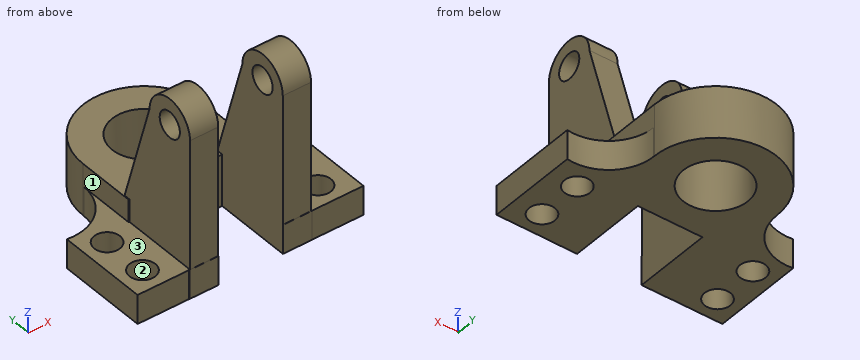
from build123d import *

# Parameters (mm, degrees)
HUB_BODY_SKETCH_R             = 20
HUB_BODY_DEPTH                = 32
MOUNTING_PLATE_DEPTH          = 18
SIDE_WEB_SKETCH_W             = 18
SIDE_WEB_SKETCH_H             = 48.092935693
SIDE_WEB_DEPTH                = 18
FORK_ARMS_DEPTH               = 37.5
FORK_SLOT_SKETCH_W            = 40
FORK_SLOT_SKETCH_H            = 48
FORK_SLOT_DEPTH               = 140.971425655
HUB_RELIEF_CUT_DEPTH          = 153.87903715
FORK_PIN_HOLE_SKETCH_R        = 8
FORK_PIN_HOLE_16_DEPTH        = 174.286612293
PLATE_MOUNTING_HOLES_SKETCH_R = 8
PLATE_MOUNTING_HOLES_16_DEPTH = 140.971425655


with BuildPart() as part:
    # Hub Body Sketch → Hub Body (new body)
    with BuildSketch(Plane.XY):
        with BuildLine():
            Line((-38, 36), (-38, 0))
            Line((-38, 0), (38, 0))
            Line((38, 0), (38, 36))
            ThreePointArc((38, 36), (0, 74), (-38, 36))
        make_face()
        with Locations((0, 36)):
            Circle(HUB_BODY_SKETCH_R, mode=Mode.SUBTRACT)
    extrude(amount=HUB_BODY_DEPTH)

    # Mounting Plate Sketch → Mounting Plate (add)
    with BuildSketch(Plane.XY):
        with BuildLine():
            Line((-38, -48), (-38, 35.425199961))
            ThreePointArc((-38, 35.425199961), (-47.777657825, 14.452308355), (-70, 8))
            Line((-70, 8), (-70, -48))
            Line((-70, -48), (-38, -48))
        make_face()
        with BuildLine():
            ThreePointArc((70, 8), (47.777657825, 14.452308355), (38, 35.425199961))
            Line((38, 35.425199961), (38, -48))
            Line((38, -48), (70, -48))
            Line((70, -48), (70, 8))
        make_face()
    extrude(amount=MOUNTING_PLATE_DEPTH)

    # Side Web Sketch → Side Web (add)
    with BuildSketch(Plane.XY):
        with Locations((-29, -24.046467847)):
            Rectangle(SIDE_WEB_SKETCH_W, SIDE_WEB_SKETCH_H)
        with Locations((29, -24.046467847)):
            Rectangle(SIDE_WEB_SKETCH_W, SIDE_WEB_SKETCH_H)
    extrude(amount=SIDE_WEB_DEPTH)

    # Fork Arms Sketch → Fork Arms (add, symmetric)
    with BuildSketch(Plane(origin=(0, 0, 0), x_dir=(0, 0, -1), z_dir=(1, 0, 0))):
        with BuildLine():
            Line((-98, -48), (-18, -48))
            Line((-18, -48), (-18, 8))
            Line((-18, 8), (-98, -16))
            ThreePointArc((-98, -16), (-114, -32), (-98, -48))
        make_face()
    extrude(amount=FORK_ARMS_DEPTH, both=True)

    # Fork Slot Sketch → Fork Slot (cut, through all)
    with BuildSketch(Plane(origin=(0, 0, 18), x_dir=(-1, 0, 0), z_dir=(0, 0, -1))):
        with Locations((0, -24)):
            Rectangle(FORK_SLOT_SKETCH_W, FORK_SLOT_SKETCH_H)
    extrude(amount=-FORK_SLOT_DEPTH, mode=Mode.SUBTRACT)

    # Hub Relief Sketch → Hub Relief Cut (cut, through all)
    with BuildSketch(Plane(origin=(0, 0, 0), x_dir=(-1, 0, 0), z_dir=(0, -1, 0))):
        Polygon((-20, -44.666666667), (20, -44.666666667), (20, -32), (11.078422409, -32), (-20, -32), align=None)
    extrude(amount=-HUB_RELIEF_CUT_DEPTH, mode=Mode.SUBTRACT)

    # Fork Pin Hole Sketch → Fork Pin Hole Ø16 (cut, through all)
    with BuildSketch(Plane.ZY.offset(37.5)):
        with Locations((98, -32)):
            Circle(FORK_PIN_HOLE_SKETCH_R)
    extrude(amount=-FORK_PIN_HOLE_16_DEPTH, mode=Mode.SUBTRACT)

    # Plate Mounting Holes Sketch → Plate Mounting Holes Ø16 (cut, through all)
    with BuildSketch(Plane.XY.offset(18)):
        with Locations((-56.00649608, -6)):
            Circle(PLATE_MOUNTING_HOLES_SKETCH_R)
        with Locations((-56.00649608, -34)):
            Circle(PLATE_MOUNTING_HOLES_SKETCH_R)
        with Locations((52.812642943, -6)):
            Circle(PLATE_MOUNTING_HOLES_SKETCH_R)
        with Locations((52.812642943, -34)):
            Circle(PLATE_MOUNTING_HOLES_SKETCH_R)
    extrude(amount=-PLATE_MOUNTING_HOLES_16_DEPTH, mode=Mode.SUBTRACT)


solid = part.part
CAD build for the part. Positions are in the model's coordinates, mm. Face numbers are marked on the shaded views. Coordinates: 2 decimals unless noted, no trailing zeros. Write each loop counter-clockwise with the first axis right and the second up, starting at its lowest first coordinate (ties: lowest second). Pieces come first, ordered by that corner, then holes. Notation, with made-up numbers: (54, 2.25) - (107, 2.25) arc R10 cw to (107, 13.25) - close; hole circle Ø9 at (-1.5, -2.5). An arc over 180 degrees is marked (long way). Use a Markdown table: item, result. Add a question column.
Item 1: Flat gauge pins, fed straight in: pin 1 (9 mm diameter, centred on x = 30, z = 68, fed in from -Y); pin 2 (1.5 mm diameter, centred on y = -12.5, z = 74, fed in from +X); pin 3 (0.6 mm diameter, centred on x = 38, z = 25.5, fed in from -Y). Where does each tip first touch, or does it go through?
Item 2: Band-saw the part on A-A, the plane z = 54. Give the cut face in (x, y), and give its area (3 significant figures).
Item 3: Mould opens along X. For the marked faces 1, 2 and 3 say: pulls with the +X half, pulls with the -X half, needs draft (parallel to the pull), parting line crosses it, or undercut.
Item 4: Band-saw the part on C-C, the plane y = -32. Give the cut face in (x, z), and give its area (3 significant figures).
Item 5: Band-saw the part on D-D, the plane y = -6. Give the cut face in (x, z).
Item 6: Band-saw the part on B-B, the plane x = 0. Give the cut face in (y, z).
Item 7: Drill centre lines: L1, parallel to X at y = -32, z = 65; L2, parallel to Y at x = 0, z = 15; L3, parallel to X at y = 36, z = 18. Where is each one in solid material? Low to high. Write a range as from..to.
Numbers:
| question | item | result |
|---|---|---|
| 1 | pin 1 | y = -48 |
| 1 | pin 2 | x = 37.5 |
| 1 | pin 3 | y = 0 |
| 2 | outline | (-37.5, -48) - (-20, -48) - (-20, -2.8) - (-37.5, -2.8) - close; (20, -48) - (37.5, -48) - (37.5, -2.8) - (20, -2.8) - close |
| 2 | area | 1,580 mm2 |
| 3 | face 1 | pulls with the -X half |
| 3 | face 2 | undercut |
| 3 | face 3 | needs draft |
| 4 | outline | (-70, 0) - (-63.75, 0) - (-63.75, 18) - (-70, 18) - close; (-48.26, 0) - (-20, 0) - (-20, 90) - (-37.5, 90) - (-37.5, 18) - (-48.26, 18) - close; (-37.5, 106) - (-20, 106) - (-20, 114) - (-37.5, 114) - close; (20, 0) - (45.07, 0) - (45.07, 18) - (37.5, 18) - (37.5, 90) - (20, 90) - close; (20, 106) - (37.5, 106) - (37.5, 114) - (20, 114) - close; (60.56, 0) - (70, 0) - (70, 18) - (60.56, 18) - close |
| 4 | area | 4,040 mm2 |
| 5 | outline | (-70, 0) - (-64.01, 0) - (-64.01, 18) - (-70, 18) - close; (-48.01, 0) - (-20, 0) - (-20, 64.67) - (-37.5, 64.67) - (-37.5, 18) - (-48.01, 18) - close; (20, 0) - (44.81, 0) - (44.81, 18) - (37.5, 18) - (37.5, 64.67) - (20, 64.67) - close; (60.81, 0) - (70, 0) - (70, 18) - (60.81, 18) - close |
| 6 | outline | (0, 0) - (16, 0) - (16, 32) - (0, 32) - close; (56, 0) - (74, 0) - (74, 32) - (56, 32) - close |
| 7 | L1 | -37.5..-20, 20..37.5 |
| 7 | L2 | 0..16, 56..74 |
| 7 | L3 | -38..-20, 20..38 |
